```python
from build123d import *

# Parameters (mm, degrees)
SKETCH_1_R             = 38
SKETCH_1_R_2           = 32.5
EXTRUDE_1_DEPTH        = 140
CHAMFER_1_SIZE         = 1
CUT_EXTRUDE_START      = -23
SKETCH_2_R             = 38
SKETCH_2_R_2           = 36.5
CUT_EXTRUDE_1_DEPTH    = 23
PATTERN_LINEAR_1_COUNT = 3
PATTERN_LINEAR_1_PITCH = 40
CHAMFER_2_SIZE         = 1


with BuildPart() as part:
    # 草图1 → 凸台-拉伸1 (new body)
    with BuildSketch(Plane.XY):
        Circle(SKETCH_1_R)
        Circle(SKETCH_1_R_2, mode=Mode.SUBTRACT)
    extrude(amount=EXTRUDE_1_DEPTH)

    # 倒角1
    chamfer_1_edges = [part.edges().sort_by_distance(p)[0] for p in [
        (-38, 0, 140),
    ]]
    chamfer(chamfer_1_edges, length=CHAMFER_1_SIZE)

    # 草图2 → 切除-拉伸1 (cut)
    with BuildSketch(Plane.XY.offset(110).offset(CUT_EXTRUDE_START)):
        Circle(SKETCH_2_R)
        Circle(SKETCH_2_R_2, mode=Mode.SUBTRACT)
    cut_extrude_1 = extrude(amount=CUT_EXTRUDE_1_DEPTH, mode=Mode.SUBTRACT)

    # 阵列(线性)1: 切除-拉伸1 ×3
    with Locations(*[(0, 0, -i * PATTERN_LINEAR_1_PITCH) for i in range(1, PATTERN_LINEAR_1_COUNT)]):
        add(cut_extrude_1, mode=Mode.SUBTRACT)

    # 倒角2
    chamfer_2_edges = [part.edges().sort_by_distance(p)[0] for p in [
        (-38, 0, 87),
        (-38, 0, 110),
        (-38, 0, 0),
        (-38, 0, 47),
        (-38, 0, 70),
        (-36.5, 0, 7),
        (-38, 0, 30),
    ]]
    chamfer(chamfer_2_edges, length=CHAMFER_2_SIZE)


solid = part.part
```
CAD build for the part. Positions are in the model's coordinates, mm. A direction names the side the tool comes from. Round coordinates to 2 decimals unless told otherwise and drop trailing zeros. Loops run counter-clockwise (first coordinate to the right, second up) from the corner with the lowest first, then second, coordinate; pieces in that order, holes last. Notation, with made-up numbers: (18.5, 2.5) - (44.5, 2.5) arc R25 cw to (44.5, 27.5) - close; hole circle Ø1 at (-24, 11). An arc over 180 degrees is marked (long way). Return JSON: item names as keys, results as strings. Group by question number.
Q1. Two-plate mould, pull along Y, no slides. Class faces 1 (the face through (0, -33, 140)), 2 (the face through (31, 9.76, 69.02)), 3 (the face through (-7.912, -35.632, 98.339)): +Y half, -Y half, draft (parallel to the pull), parting line (faces both ways), or undercut.
Q2. Band-saw the part on B-B on z = 34.5. Give the cut face in (x, y).
Q3. Drill centre lines: line 1 along Y through (x, z) = (0, 82.5); line 2 along X through (y, z) = (1, 12); line 3 along Y through (x, z) = (10, 36.5). Where is each one in solid material? Low to high. Write a range as [from, to].
Q4. Band-saw the part on A-A on z = 12.5. Give the cut face in (x, y).
Q5. Flat gauge pins, fed straight in: pin 1 Ø12 at (y, z) = (25, 56.5) entering from +X; pin 2 Ø1 at (x, z) = (-6.5, 22) entering from +Y; pin 3 Ø12 at (x, z) = (-3.5, 24.5) entering from +Y. Where does each tip first touch, or does it go through?
Q6. Tool access for faces 4 (the face through (-7.912, -35.632, 58.339)), 5 (the face through (17.535, -33.713, 124.804)): list every direction of +Z, -Z, +X, -X, +Y, -Y with a clear straight run to the whole face (end or side of a thin tool).
Solutions:
{
 "1": {"face 1": "draft", "face 2": "undercut", "face 3": "parting line"},
 "2": {"outline": "circle Ø76 at (0, 0); hole circle Ø65 at (0, 0)"},
 "3": {"line 1": "y = [-38, -32.5], [32.5, 38]", "line 2": "x = [-36.49, -32.48], [32.48, 36.49]", "line 3": "y = [-36.66, -30.92], [30.92, 36.66]"},
 "4": {"outline": "circle Ø73 at (0, 0); hole circle Ø65 at (0, 0)"},
 "5": {"pin 1": "stops at x = 31.16", "pin 2": "stops at y = 36", "pin 3": "stops at y = 37.36"},
 "6": {"face 4": "none", "face 5": "+Z, -Z"}
}
